```python
from build123d import *

# Parameters (mm, degrees)
HEX_HEAD_DEPTH    = 3
SHANK_PROFILE_6_R = 3
SHANK_6X12_DEPTH  = 12


with BuildPart() as part:
    # Hex Head Profile 10AF → Hex Head (new body)
    with BuildSketch(Plane.XY):
        Polygon((-2.886751346, 5), (-5.773502692, 0), (-2.886751346, -5), (2.886751346, -5), (5.773502692, 0), (2.886751346, 5), align=None)
    extrude(amount=HEX_HEAD_DEPTH)

    # Shank Profile Ø6 → Shank Ø6x12 (add)
    with BuildSketch(Plane.XY.offset(3)):
        Circle(SHANK_PROFILE_6_R)
    extrude(amount=SHANK_6X12_DEPTH)

    # Head Chamfer Profile → Head Chamfer 45x1 (revolve, cut)
    with BuildSketch(Plane(origin=(0, 0, 0), x_dir=(1, 0, 0), z_dir=(0, 1, 0)), mode=Mode.PRIVATE) as head_chamfer_45x1_sk:
        Polygon((-4.773502692, 0), (-5.773502692, 0), (-5.773502692, -1), align=None)
    revolve(head_chamfer_45x1_sk.sketch.rotate(Axis((0, 0, -2.775923962), (0, 0, 1)), 180), axis=Axis((0, 0, -2.775923962), (0, 0, 1)), mode=Mode.SUBTRACT)


solid = part.part
```
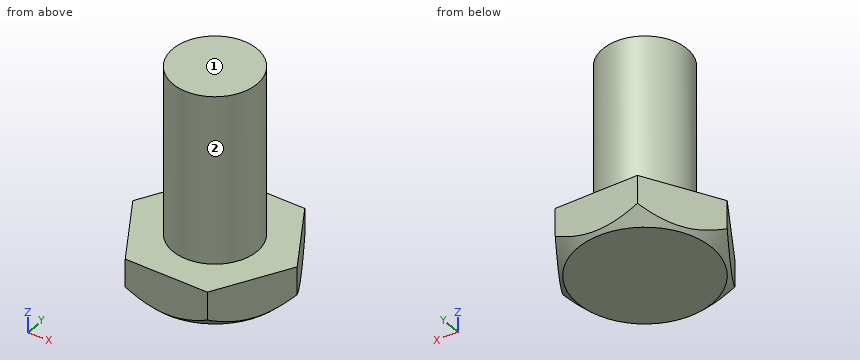
Geometry check sheet. Reference: the model listing, model coordinates, mm. Face numbers are marked on the shaded views. A direction names the side the tool comes from. Coordinates: 2 decimals unless noted, no trailing zeros. Write each loop counter-clockwise with the first axis right and the second up, starting at its lowest first coordinate (ties: lowest second). Pieces come first, ordered by that corner, then holes. Notation, with made-up numbers: M 40.5,57.25 L 88.5,57.25 A31 ccw 88.5,83.25 Z; hole C 25.25,86 d7. An arc over 180 degrees is marked long. One line per item, written item: value. Start each with the question number.
(1) Sectioned sample at A-A, the plane x = 0. Enter the section's corners in (y, z), and give its area (3 significant figures).
(2) Tool access check on the marked faces 1 and 2. Record the directions out of +Z, -Z, +X, -X, +Y, -Y that give a thin tool (end or side, any length) a straight path to the whole face; none if there is none.
(3) Sectioned sample at B-B, the plane z = 12.5. Enter the section's corners in (x, y), and give its area (3 significant figures).
(4) Depth check by flat-ended pin: pin 1 (1.5 mm diameter, centred on y = 3, z = 9, fed in from -X); pin 2 (3 mm diameter, centred on y = 4, z = 4, fed in from +X); pin 3 (1.5 mm diameter, centred on y = 3.5, z = 4.5, fed in from -X). Enter the tip coordinate at first touch or a pass-through.
(5) Scan lines: line 1 along Z through (x, y) = (-2.5, 2.5); line 2 along Z through (x, y) = (-3, 4); line 3 along X through (y, z) = (-1.75, 10.5). Record each from-to range of solid material in increasing order. Write a range as [from, to].
Filled sheet:
1. outline: M -5,0.23 L -4.77,0 L 4.77,0 L 5,0.23 L 5,3 L 3,3 L 3,15 L -3,15 L -3,3 L -5,3 Z
1. area: 102 mm²
2. face 1: +Z, +X, -X, +Y, -Y
2. face 2: +Z
3. outline: C 0,0 d6
3. area: 28.3 mm²
4. pin 1: x = -1.98
4. pin 2: x = 4.11
4. pin 3: x = -1.2
5. line 1: [0, 3]
5. line 2: [0.23, 3]
5. line 3: [-2.44, 2.44]
